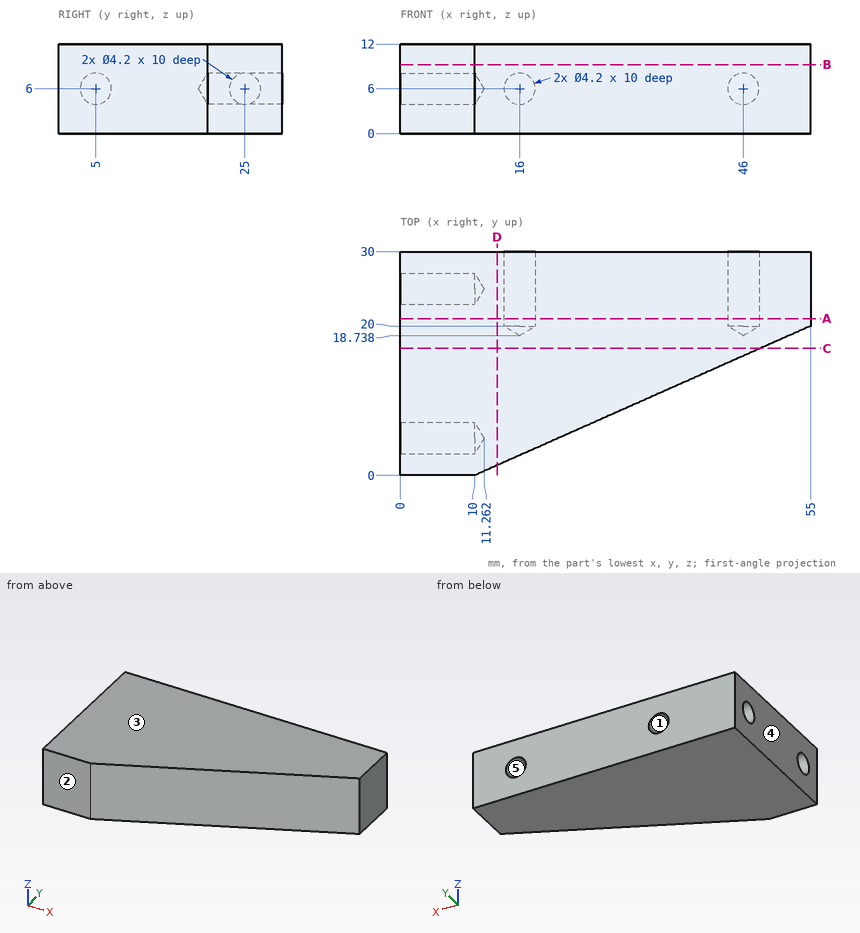
Study the drawing (mm; zero at the part's minimum x, y, z) and answer. A direction names the side the tool comes from. Coordinates: 2 decimals unless noted, no trailing zeros. Write each loop counter-clockwise with the first axis right and the second up, starting at its lowest first coordinate (ties: lowest second). Pieces come first, ordered by that corner, then holes. Notation, with made-up numbers: (22.25, 83) - (58.25, 83) arc R28 ccw to (58.25, 117) - close; hole circle Ø5 at (-16, 56.25). An arc over 180 degrees is marked (long way). Answer as a JSON object with one key per item and string values.
Q1. Which of the six approach directions +Z, -Z, +X, -X, +Y, -Y give full straight-line access (tool end or side, diameter ignored) to the marked faces 1 and 2?
Results list:
{"face 1": "+Y", "face 2": "+Z, -Z, +X, -X, -Y"}
Q2. Given pin 1 Ø3 at (x, z) = (33, 6.5) entering from -Y; pin 2 Ø3.5 at (x, z) = (16, 6) entering from -Y; pin 3 Ø4 at (y, z) = (5, 6) entering from +X, each flat-ended and moving along its own axis, determine where each tip first touches the part or whether it passes through.
Results list:
{"pin 1": "stops at y = 9.56", "pin 2": "stops at y = 1.89", "pin 3": "stops at x = 25.75"}
Q3. For a pull along Z with two mould halves and no side action, classify the marked faces 3, 4 and 5 as pulls with the +Z half, pulls with the -Z half, needs draft (parallel to the pull), parting line crosses it, or undercut.
Results list:
{"face 3": "pulls with the +Z half", "face 4": "needs draft", "face 5": "undercut"}
Q4. Find section C-C (y = 17). Write down the section's boundary in (x, z).
Results list:
{"outline": "(0, 0) - (48.25, 0) - (48.25, 12) - (0, 12) - close"}
Q5. Find section D-D (x = 13). Write down the section's boundary in (y, z), plus the area to 3 significant figures.
Results list:
{"outline": "(1.33, 0) - (30, 0) - (30, 12) - (1.33, 12) - close", "area": "344 mm^2"}
Q6. Consider L1, parallel to Y at x = 6, z = 6; L2, parallel to Z at x = 6, y = 25; L3, parallel to X at y = 25, z = 6.5. Determine where each line is inside the solid, lowest interval first. Write a range as from..to.
Results list:
{"L1": "y = 0..2.9, 7.1..22.9, 27.1..30", "L2": "z = 0..3.9, 8.1..12", "L3": "x = 10.96..13.96, 18.04..43.96, 48.04..55"}
Q7. Find section B-B (z = 9.25). Write down the section's boundary in (x, y).
Results list:
{"outline": "(0, 0) - (10, 0) - (55, 20) - (55, 30) - (0, 30) - close"}
Q8. Find section A-A (y = 21). Write down the section's boundary in (x, z), plus the area to 3 significant figures.
Results list:
{"outline": "(0, 0) - (55, 0) - (55, 12) - (0, 12) - close; hole circle Ø4.2 at (16, 6); hole circle Ø4.2 at (46, 6)", "area": "632 mm^2"}
